Could you check a few things on this model? Use its own coordinates, in mm. Round coordinates to 2 decimals unless told otherwise and drop trailing zeros. Loops run counter-clockwise (first coordinate to the right, second up) from the corner with the lowest first, then second, coordinate; pieces in that order, holes last.
from build123d import *

# Parameters (mm, degrees)
EXTRUDE_1_DEPTH = 8
CHAMFER_1_SIZE  = 20


with BuildPart() as part:
    # 草图2 → 凸台-拉伸1 (new, symmetric)
    with BuildSketch(Plane.XY):
        Polygon((25, 90), (66, 90), (66, 0), (0, 0), (0, 38), align=None)
    extrude(amount=EXTRUDE_1_DEPTH, both=True)

    # 倒角1
    chamfer_1_edges = [part.edges().sort_by_distance(p)[0] for p in [
        (66, 0, 0),
    ]]
    chamfer(chamfer_1_edges, length=CHAMFER_1_SIZE)


solid = part.part
Item 1: If I drill on line 1 along X through (y, z) = (60, -1.25); line 2 along X through (y, z) = (70.5, -7) (3 decimals); line 3 along Y through (x, z) = (21.5, 3.25), over which ranges is the centre line in solid material (lowest first)?
Results list:
line 1: x = 10.58 to 66
line 2: x = 15.625 to 66
line 3: y = 0 to 82.72
Item 2: If we section it at B-B, the plane y = 7.5: Please give me the cut outline in (x, z), then the cut area to 3 significant figures.
Results list:
outline: (0, -8) - (53.5, -8) - (53.5, 8) - (0, 8) - close
area: 856 mm2
Item 3: Will this pin go through, and if not, where does the flat tip stop? pin 1 (1 mm diameter, centred on y = 50, z = -5, fed in from -X).
Results list:
pin 1: stops at x = 5.53
Item 4: If we section it at A-A, the plane z = -4.5: Please give me the cut outline in (x, y), then the cut area to 3 significant figures.
Results list:
outline: (0, 0) - (46, 0) - (66, 20) - (66, 90) - (25, 90) - (0, 38) - close
area: 5,090 mm2
Item 5: If we section it at C-C, the plane x = 48.5: Please give me the cut outline in (y, z).
Results list:
outline: (2.5, -8) - (90, -8) - (90, 8) - (2.5, 8) - close
